Here's how the part is built. I have some questions about the finished solid (model axes, mm). A direction names the side the tool comes from. Coordinates: 2 decimals unless noted, no trailing zeros. Write each loop counter-clockwise with the first axis right and the second up, starting at its lowest first coordinate (ties: lowest second). Pieces come first, ordered by that corner, then holes. Notation, with made-up numbers: (65.25, -3) -> (84.25, -3) arc R14 cw to (84.25, 19) -> close; hole circle Ø5 at (55, 13). An arc over 180 degrees is marked (long way). Put each result on its own line as item: value.
```python
from build123d import *

# Parameters (mm, degrees)
EXTRUDE_2_DEPTH = 100


with BuildPart() as part:
    # 草图1 → 凸台-拉伸2 (new body)
    with BuildSketch(Plane.XY):
        Polygon((0, 0), (30, 0), (30, 30), (28, 30), (28, 2), (0, 2), align=None)
    extrude(amount=EXTRUDE_2_DEPTH)


solid = part.part
```
Item 1: Which directions (+Z, -Z, +X, -X, +Y, -Y) give clear straight access to the entire face, cutting with the end or side of a thin tool? Please do faces 1 (the flat face through (21.6, 1.7, 0)), 2 (the flat face through (14, 2, 49)).
Output:
face 1: -Z, +X, -X, +Y, -Y
face 2: +Z, -Z, -X, +Y
Item 2: Please list where these lines run through material, in increasing order: line 1 along Y through (x, z) = (15, 83.5); line 2 along X through (y, z) = (5.5, 73.5). Write a range as from..to.
Output:
line 1: y = 0..2
line 2: x = 28..30
Item 3: Imagine slicing it at B-B on x = 9. Write out the boundary of the cut face in (y, z).
Output:
outline: (0, 0) -> (2, 0) -> (2, 100) -> (0, 100) -> close
Item 4: For P1, Ø1.5, axis at y = 18.5, z = 23, coming from the -X side; P2, Ø3, axis at x = 13, z = 26, coming from the +Y side, each with a flat end and sliding along its axis, tell me the tip position at first contact or that it passes through.
Output:
P1: stops at x = 28
P2: stops at y = 2
Item 5: Imagine slicing it at A-A on z = 88. Write out the boundary of the cut face in (x, y), then the cut area to 3 significant figures.
Output:
outline: (0, 0) -> (30, 0) -> (30, 30) -> (28, 30) -> (28, 2) -> (0, 2) -> close
area: 116 mm²
Item 6: Imagine slicing it at C-C on y = 6. Write out the boundary of the cut face in (x, z), then the cut area to 3 significant figures.
Output:
outline: (28, 0) -> (30, 0) -> (30, 100) -> (28, 100) -> close
area: 200 mm²
